Can you work these out from the model? Positions are in its coordinate system, mm. Face numbers are marked on the shaded views. A direction names the side the tool comes from. Round coordinates to 2 decimals unless told otherwise and drop trailing zeros. Loops run counter-clockwise (first coordinate to the right, second up) from the corner with the lowest first, then second, coordinate; pieces in that order, holes last. Notation, with made-up numbers: (45.25, 85) - (57.25, 85) arc R22 cw to (57.25, 105) - close; hole circle Ø6 at (38.5, -15). An arc over 180 degrees is marked (long way). Answer as CSV lines item,"result".
```python
from build123d import *

# Parameters (mm, degrees)
SKETCH1_W                                           = 75
SKETCH1_H                                           = 60
BOSS_EXTRUDE1_DEPTH                                 = 6
M6_TAPPED_HOLE1_D                                   = 5
CBORE_FOR_M6_HEX_SOCKET_HEAD_CAP_SCREW1_D           = 6.6
CBORE_FOR_M6_HEX_SOCKET_HEAD_CAP_SCREW1_CBORE_D     = 11
CBORE_FOR_M6_HEX_SOCKET_HEAD_CAP_SCREW1_CBORE_DEPTH = 6.4
BLIND_PIN_HOLE3_SIZE_MM_D                           = 5
BLIND_PIN_HOLE3_SIZE_MM_DEPTH                       = 11
BLIND_PIN_HOLE3_SIZE_MM_TIP                         = 1.502151548
MM_3_D                                              = 5
MM_3_DEPTH                                          = 10
MM_3_TIP                                            = 1.502151548
CHAMFER1_SIZE                                       = 1


with BuildPart() as part:
    # Sketch1 → Boss-Extrude1 (new, symmetric)
    with BuildSketch(Plane.XY):
        Rectangle(SKETCH1_W, SKETCH1_H)
    extrude(amount=BOSS_EXTRUDE1_DEPTH, both=True)

    # M6 Tapped Hole1 (through all)
    with Locations(Plane.XY.offset(6)):
        with Locations((30, 24), (30, -24), (-30, -24), (-30, 24)):
            Hole(M6_TAPPED_HOLE1_D / 2)

    # CBORE for M6 Hex Socket Head Cap Screw1 (through all)
    with Locations(Plane.XY.offset(6)):
        with Locations((-30, 12.5), (30, 12.5), (-30, -12.5), (30, -12.5)):
            CounterBoreHole(CBORE_FOR_M6_HEX_SOCKET_HEAD_CAP_SCREW1_D / 2, CBORE_FOR_M6_HEX_SOCKET_HEAD_CAP_SCREW1_CBORE_D / 2, CBORE_FOR_M6_HEX_SOCKET_HEAD_CAP_SCREW1_CBORE_DEPTH)

    # Blind Pin Hole3 (size mm)
    with Locations(Plane.XY.offset(6)):
        with Locations((-30, 0), (30, 0)):
            Hole(BLIND_PIN_HOLE3_SIZE_MM_D / 2, depth=BLIND_PIN_HOLE3_SIZE_MM_DEPTH)
            with Locations((0, 0, -(BLIND_PIN_HOLE3_SIZE_MM_DEPTH + BLIND_PIN_HOLE3_SIZE_MM_TIP / 2))):  # 118° drill point
                Cone(0, BLIND_PIN_HOLE3_SIZE_MM_D / 2, BLIND_PIN_HOLE3_SIZE_MM_TIP, mode=Mode.SUBTRACT)

    # 大小mm 暗销孔3
    with Locations(Plane.XY.offset(6)):
        with Locations((-15, 24), (15, -24), (15, 24), (-15, -24)):
            Hole(MM_3_D / 2, depth=MM_3_DEPTH)
            with Locations((0, 0, -(MM_3_DEPTH + MM_3_TIP / 2))):  # 118° drill point
                Cone(0, MM_3_D / 2, MM_3_TIP, mode=Mode.SUBTRACT)

    # Chamfer1
    chamfer1_edges = [part.edges().sort_by_distance(p)[0] for p in [
        (37.5, -30, 0),
        (-37.5, -30, 0),
        (-37.5, 30, 0),
        (37.5, 30, 0),
    ]]
    chamfer(chamfer1_edges, length=CHAMFER1_SIZE)


solid = part.part
```
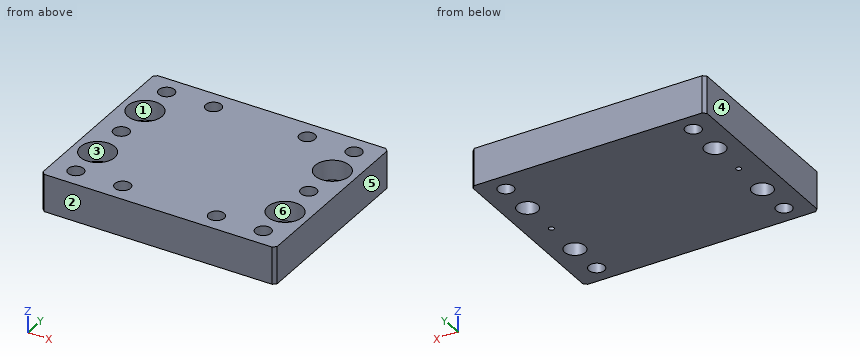
Q1. I'm going to push flat-ended pins straight in: pin 1 Ø4 at (x, y) = (-30, -12.5) entering from +Z; pin 2 Ø9 at (x, y) = (-30, 12.5) entering from +Z; pin 3 Ø3 at (x, y) = (-15, -24) entering from +Z. Where does each tip first touch, or does it pass through?
Checks:
pin 1,"through"
pin 2,"z = -0.4"
pin 3,"z = -4.6"
Q2. Imagine slicing it at A-A (y = -12.5). Write out the boundary of the cut face in (x, z).
Checks:
outline,"(-37.5, -6) - (-33.3, -6) - (-33.3, -0.4) - (-35.5, -0.4) - (-35.5, 6) - (-37.5, 6) - close; (-26.7, -6) - (26.7, -6) - (26.7, -0.4) - (24.5, -0.4) - (24.5, 6) - (-24.5, 6) - (-24.5, -0.4) - (-26.7, -0.4) - close; (33.3, -6) - (37.5, -6) - (37.5, 6) - (35.5, 6) - (35.5, -0.4) - (33.3, -0.4) - close"
Q3. Imagine slicing it at B-B (z = 1.5). Count the separate pieces of the cut face and the enclosed holes in it, then the cut area to 3 significant figures.
Checks:
separate pieces,"1"
enclosed holes,"14"
area,"3,920 mm²"
Q4. If I drill on line 1 along Y through (x, z) = (-15, 0.25); line 2 along Y through (x, z) = (-30, -2.35); line 3 along Y through (x, z) = (-14, -3), over which ranges is the centre line in solid material (lowest first)? Write a range as [from, to].
Checks:
line 1,"[-30, -26.5], [-21.5, 21.5], [26.5, 30]"
line 2,"[-30, -26.5], [-21.5, -15.8], [-9.2, -2.5], [2.5, 9.2], [15.8, 21.5], [26.5, 30]"
line 3,"[-30, -26.29], [-21.71, 21.71], [26.29, 30]"
Q5. We'd pull the mould along X, two halves only. Please class the marked faces 3, 4, 5 and 6: pulls with the +X half, pulls with the -X half, needs draft (parallel to the pull), parting line crosses it, or undercut.
Checks:
face 3,"undercut"
face 4,"pulls with the -X half"
face 5,"pulls with the +X half"
face 6,"undercut"
Q6. On a 3-axis mill with a long thin cutter (end or side, diameter ignored), from which of +Z, -Z, +X, -X, +Y, -Y can I reach the whole of each face in a straight line? I mean the marked faces 1 and 2. Say none if no direction works.
Checks:
face 1,"+Z"
face 2,"+Z, -Z, +X, -X, -Y"
